from build123d import *

# Parameters (mm, degrees)
EXTRUDE_THIN2_DEPTH = 58
SKETCH2_R           = 2.5
CUT_EXTRUDE1_DEPTH  = 10
CUT_EXTRUDE2_DEPTH  = 10


with BuildPart() as part:
    # Sketch1 → Extrude-Thin2 (new body)
    with BuildSketch(Plane.XY):
        Polygon((0, 0), (0, -34), (-19.5, -275), (-25, -280), (-30, -280), (-30, -281.5), (-24.420089688, -281.5), (-18.0526616, -275.711429011), (1.5, -34.060585647), (1.5, 0), align=None)
    extrude(amount=EXTRUDE_THIN2_DEPTH)

    # Sketch2 → Cut-Extrude1 (cut)
    with BuildSketch(Plane(origin=(1.5, 0, 0), x_dir=(0, 0, -1), z_dir=(1, 0, 0))):
        with Locations(Location((-14, -7, 0), (0, 0, 90))):
            Circle(SKETCH2_R)
        with Locations(Location((-44, -7, 0), (0, 0, 90))):
            Circle(SKETCH2_R)
    extrude(amount=-CUT_EXTRUDE1_DEPTH, mode=Mode.SUBTRACT)

    # Sketch3 → Cut-Extrude2 (cut)
    with BuildSketch(Plane(origin=(4.228257559, -0.342120425, 0), x_dir=(0, 0, -1), z_dir=(0.9967425402733565, -0.08064929267772025, 0))):
        with BuildLine():
            Line((-51.5, -97.379026061), (-51.5, -102.379026061))
            ThreePointArc((-51.5, -102.379026061), (-54, -104.879026061), (-56.5, -102.379026061))
            Line((-56.5, -102.379026061), (-56.5, -97.379026061))
            ThreePointArc((-56.5, -97.379026061), (-54, -94.879026061), (-51.5, -97.379026061))
        make_face()
        with BuildLine():
            Line((-51.5, -262.379026061), (-51.5, -257.379026061))
            ThreePointArc((-51.5, -257.379026061), (-54, -254.879026061), (-56.5, -257.379026061))
            Line((-56.5, -257.379026061), (-56.5, -262.379026061))
            ThreePointArc((-56.5, -262.379026061), (-54, -264.879026061), (-51.5, -262.379026061))
        make_face()
    cut_extrude2 = extrude(amount=-CUT_EXTRUDE2_DEPTH, mode=Mode.SUBTRACT)

    # Mirror1: Cut-Extrude2 across plane
    add(cut_extrude2.mirror(Plane.XY.offset(29)), mode=Mode.SUBTRACT)


solid = part.part
Build history of the part. All positions in model axes, mm. A direction names the side the tool comes from. Round coordinates to 2 decimals unless told otherwise and drop trailing zeros. Loops run counter-clockwise (first coordinate to the right, second up) from the corner with the lowest first, then second, coordinate; pieces in that order, holes last. Notation, with made-up numbers: (-4.75, 28.25) -> (18.25, 28.25) arc R17 ccw to (18.25, 58.25) -> close; hole circle Ø3 at (-28, 51). An arc over 180 degrees is marked (long way). Answer in a Markdown table with one row per item.
Item 1: Saw through at D-D (x = -12). Write the cut outline in (y, z), and give its area (3 significant figures).
Answers below:
| item | result |
|---|---|
| outline | (-200.91, 0) -> (-182.31, 0) -> (-182.31, 58) -> (-200.91, 58) -> close |
| area | 1,080 mm² |
Item 2: Saw through at C-C (z = 49). Write the cut outline in (x, y), and give its area (3 significant figures).
Answers below:
| item | result |
|---|---|
| outline | (-30, -281.5) -> (-24.42, -281.5) -> (-18.05, -275.71) -> (1.5, -34.06) -> (1.5, 0) -> (0, 0) -> (0, -34) -> (-19.5, -275) -> (-25, -280) -> (-30, -280) -> close |
| area | 434 mm² |
Item 3: Saw through at B-B (y = -7). Write the cut outline in (x, z).
Answers below:
| item | result |
|---|---|
| outline | (0, 0) -> (1.5, 0) -> (1.5, 11.5) -> (0, 11.5) -> close; (0, 16.5) -> (1.5, 16.5) -> (1.5, 41.5) -> (0, 41.5) -> close; (0, 46.5) -> (1.5, 46.5) -> (1.5, 58) -> (0, 58) -> close |
Item 4: Pin check, flat tips, straight feed: pin 1 (2.5 mm diameter, centred on x = -27, z = 24.5, fed in from +Y); pin 2 (10 mm diameter, centred on y = -9.5, z = 31.5, fed in from -X); pin 3 (1 mm diameter, centred on y = -210.5, z = 47, fed in from +X). Stop position of each tip, or through.
Answers below:
| item | result |
|---|---|
| pin 1 | stops at y = -280 |
| pin 2 | stops at x = 0 |
| pin 3 | stops at x = -12.74 |
Item 5: Saw through at A-A (z = 14). Write the cut outline in (x, y), and give its area (3 significant figures).
Answers below:
| item | result |
|---|---|
| outline | (-30, -281.5) -> (-24.42, -281.5) -> (-18.05, -275.71) -> (1.5, -34.06) -> (1.5, -9.5) -> (0, -9.5) -> (0, -34) -> (-19.5, -275) -> (-25, -280) -> (-30, -280) -> close; (0, -4.5) -> (1.5, -4.5) -> (1.5, 0) -> (0, 0) -> close |
| area | 427 mm² |
Item 6: Which spindle directions (+Z, -Z, +X, -X, +Y, -Y) get a long thin tool onto all of the face, cutting with end or side? Do faces 1 (the flat face through (0, -17, 29)), 2 (the flat face through (-8.5, -150.5, 0)). Say none if no direction does.
Answers below:
| item | result |
|---|---|
| face 1 | +Z, -Z, -X, +Y |
| face 2 | -Z, +X, -X, +Y, -Y |
Item 7: Drill centre lines: L1, parallel to Z at x = 1, y = -7; L2, parallel to X at y = -93.5, z = 10; L3, parallel to X at y = -176, z = 41.5. Where is each one in solid material? Low to high. Write a range as [from, to].
Answers below:
| item | result |
|---|---|
| L1 | z = [0, 11.5], [16.5, 41.5], [46.5, 58] |
| L2 | x = [-4.81, -3.31] |
| L3 | x = [-11.49, -9.98] |
Item 8: Mould opens along Z. For faces 3 (the flat face through (-8.5, -150.5, 58)), 4 (the flat face through (-27, -280, 29)), 5 (the cylindrical face through (0.76, -5.85, 11.78)) say: +Z half, -Z half, draft (parallel to the pull), parting line (faces both ways), or undercut.
Answers below:
| item | result |
|---|---|
| face 3 | +Z half |
| face 4 | draft |
| face 5 | undercut |
